```python
from build123d import *

# Parameters (mm, degrees)
SKETCH1_W           = 129
SKETCH1_H           = 210
SKETCH1_R           = 3
SKETCH1_W_2         = 99
SKETCH1_H_2         = 180
BOSS_EXTRUDE1_DEPTH = 1
SCALE_1_SCALE       = 1.875


with BuildPart() as part:
    # Sketch1 → Boss-Extrude1 (new body)
    with BuildSketch(Plane(origin=(0, 0, 0), x_dir=(1, 0, 0), z_dir=(0, 1, 0))):
        with Locations((23.903865936, 105)):
            Rectangle(SKETCH1_W, SKETCH1_H)
        with Locations(Location((-32.596134064, 8, 0), (0, 0, 270))):
            Circle(SKETCH1_R, mode=Mode.SUBTRACT)
        with Locations(Location((81.403865936, 8, 0), (0, 0, 270))):
            Circle(SKETCH1_R, mode=Mode.SUBTRACT)
        with Locations(Location((81.403865936, 202, 0), (0, 0, 270))):
            Circle(SKETCH1_R, mode=Mode.SUBTRACT)
        with Locations(Location((-32.596134064, 202, 0), (0, 0, 270))):
            Circle(SKETCH1_R, mode=Mode.SUBTRACT)
        with Locations((23.903865936, 105)):
            Rectangle(SKETCH1_W_2, SKETCH1_H_2, mode=Mode.SUBTRACT)
    extrude(amount=BOSS_EXTRUDE1_DEPTH)


with BuildPart() as part_1:
    # Scale 1: scaled about (23.897690412, 0.5, -105)
    add(part.part.scale(SCALE_1_SCALE).moved(Location((-20.91047911, -0.4375, 91.875))))


solid = part_1.part
```
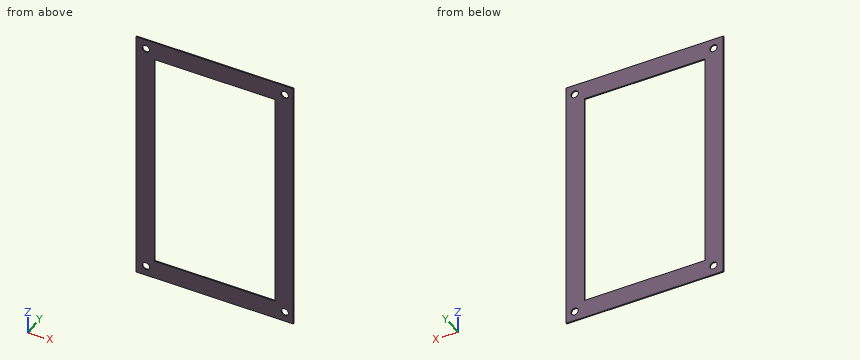
Source: CAD feature listing. Evaluate the final solid. Frame: model axes, mm. Coordinates: 2 decimals unless noted, no trailing zeros. Loops run counter-clockwise (first coordinate to the right, second up) from the corner with the lowest first, then second, coordinate; pieces in that order, holes last. Notation, with made-up numbers: (24, 53) -> (42, 53) arc R11 cw to (42, 65) -> close; hole circle Ø2 at (70.5, 62). An arc over 180 degrees is marked (long way). One line per item, written item: value. Start each with the question number.
Q1. Section query C-C, the plane y = 0. Return the cut outline in (x, z) (3 decimals).
Q2. Section query B-B, the plane z = -229.5. Return the cut outline in (x, y).
Q3. Line query: line 1 along Z through (x, y) = (131.5, 0.1) (3 decimals); line 2 along X through (y, z) = (1.15, -203); line 3 along Z through (x, y) = (73, -0.25) (3 decimals). Output: solid intervals per line, ascending.
Results:
1. outline: (-97.028, -301.875) -> (144.847, -301.875) -> (144.847, 91.875) -> (-97.028, 91.875) -> close; hole circle Ø11.25 at (-82.028, -286.875); hole circle Ø11.25 at (-82.028, 76.875); hole (-68.903, -273.75) -> (116.722, -273.75) -> (116.722, 63.75) -> (-68.903, 63.75) -> close; hole circle Ø11.25 at (131.722, -286.875); hole circle Ø11.25 at (131.722, 76.875)
2. outline: (-97.03, -0.44) -> (-68.9, -0.44) -> (-68.9, 1.44) -> (-97.03, 1.44) -> close; (116.72, -0.44) -> (144.85, -0.44) -> (144.85, 1.44) -> (116.72, 1.44) -> close
3. line 1: -301.875 to -292.496, -281.254 to 71.254, 82.496 to 91.875
3. line 2: -97.03 to -68.9, 116.72 to 144.85
3. line 3: -301.875 to -273.75, 63.75 to 91.875
